```python
from build123d import *

# Parameters (mm, degrees)
SKETCH1_R             = 4
BOSS_EXTRUDE1_DEPTH   = 78.5
SKETCH2_R             = 2.5
BOSS_EXTRUDE2_DEPTH   = 8
CHAMFER1_SIZE         = 0.3
M4_TAPPED_HOLE1_D     = 3.3
M4_TAPPED_HOLE1_DEPTH = 10.1
M4_TAPPED_HOLE1_TIP   = 0.991420021
SKETCH6_R             = 1.75
CUT_EXTRUDE1_DEPTH    = 5
SKETCH7_W             = 0.3
SKETCH7_H             = 0.5


with BuildPart() as part:
    # Sketch1 → Boss-Extrude1 (new body)
    with BuildSketch(Plane(origin=(0, 0, 0), x_dir=(1, 0, 0), z_dir=(0, 1, 0))):
        with Locations(Location((0, 0, 0), (0, 0, 270))):
            Circle(SKETCH1_R)
    extrude(amount=BOSS_EXTRUDE1_DEPTH)

    # Sketch2 → Boss-Extrude2 (add)
    with BuildSketch(Plane(origin=(0, 78.5, 0), x_dir=(1, 0, 0), z_dir=(0, 1, 0))):
        with Locations(Location((0, 0, 0), (0, 0, 270))):
            Circle(SKETCH2_R)
    extrude(amount=BOSS_EXTRUDE2_DEPTH)

    # Chamfer1
    chamfer1_edges = [part.edges().sort_by_distance(p)[0] for p in [
        (0, 0, -4),
        (0, 78.5, -4),
        (0, 86.5, -2.5),
    ]]
    chamfer(chamfer1_edges, length=CHAMFER1_SIZE)

    # M4 Tapped Hole1
    with Locations(Plane(origin=(0, 0, 0), x_dir=(-1, 0, 0), z_dir=(0, -1, 0))):
        with Locations((0, 0)):
            Hole(M4_TAPPED_HOLE1_D / 2, depth=M4_TAPPED_HOLE1_DEPTH)
            with Locations((0, 0, -(M4_TAPPED_HOLE1_DEPTH + M4_TAPPED_HOLE1_TIP / 2))):  # 118° drill point
                Cone(0, M4_TAPPED_HOLE1_D / 2, M4_TAPPED_HOLE1_TIP, mode=Mode.SUBTRACT)

    # Sketch6 → Cut-Extrude1 (cut, symmetric)
    with BuildSketch(Plane.XY):
        with Locations(Location((0, 57, 0), (0, 0, 90))):
            Circle(SKETCH6_R)
    extrude(amount=CUT_EXTRUDE1_DEPTH, both=True, mode=Mode.SUBTRACT)

    # Sketch7 → Cut-Revolve1 (revolve, cut)
    with BuildSketch(Plane.XY, mode=Mode.PRIVATE) as cut_revolve1_sk:
        with Locations((2.35, 78.75)):
            Rectangle(SKETCH7_W, SKETCH7_H)
    revolve(cut_revolve1_sk.sketch.rotate(Axis((0, 0, 0), (0, 1, 0)), 90), axis=Axis((0, 0, 0), (0, 1, 0)), mode=Mode.SUBTRACT)


solid = part.part
```
Work out the finished part from the listing and answer in its coordinate system (mm). A direction names the side the tool comes from. Coordinates: 2 decimals unless noted, no trailing zeros. Loops run counter-clockwise (first coordinate to the right, second up) from the corner with the lowest first, then second, coordinate; pieces in that order, holes last. Notation, with made-up numbers: (87.25, 48.25) - (114.25, 48.25) arc R15 ccw to (114.25, 65.25) - close; hole circle Ø4 at (10.25, 28.5). An arc over 180 degrees is marked (long way). Use a Markdown table: item, result.
Item 1: The mould has two halves that part along Z. Classify faces 1 (the cylindrical face through (-2.44, 82.55, -0.54)), 2 (the flat face through (0, 86.5, 0)), 3 (the cylindrical face through (-1.216, 5.121, -1.115)): +Z half, -Z half, draft (parallel to the pull), parting line (faces both ways), or undercut.
Evaluation:
| item | result |
|---|---|
| face 1 | parting line |
| face 2 | draft |
| face 3 | undercut |
Item 2: Find section C-C, the plane y = 8. Determine the outline of the cut face in (x, z).
Evaluation:
| item | result |
|---|---|
| outline | circle Ø8 at (0, 0); hole circle Ø3.3 at (0, 0) |
Item 3: Find section B-B, the plane y = 57. Determine the outline of the cut face in (x, z).
Evaluation:
| item | result |
|---|---|
| outline | (-1.75, -3.6) - (-1.75, 3.6) arc R4 ccw to start; (1.75, -3.6) arc R4 ccw to (1.75, 3.6) - close |
Item 4: Given pin 1 Ø3 at (x, z) = (1.5, -2) entering from -Y; pin 2 Ø1.5 at (y, z) = (27.5, 3) entering from -X; pin 3 Ø1.5 at (x, y) = (-2.5, 47) entering from -Z, each flat-ended and moving along its own axis, determine where each tip first touches the part or whether it passes through.
Evaluation:
| item | result |
|---|---|
| pin 1 | stops at y = 0 |
| pin 2 | stops at x = -3.31 |
| pin 3 | stops at z = -3.6 |
Item 5: Consider probe 1 along Y at (x, z) = (0, 2.75); probe 2 along X at (y, z) = (57, 1.5); probe 3 along Z at (x, y) = (0, 7.25). Determine where each line is inside the solid, lowest interval first. Write a range as from..to.
Evaluation:
| item | result |
|---|---|
| probe 1 | y = 0..55.25, 58.75..78.5 |
| probe 2 | x = -3.71..-1.75, 1.75..3.71 |
| probe 3 | z = -4..-1.65, 1.65..4 |
Item 6: Find section A-A, the plane y = 72. Determine the outline of the cut face in (x, z), and give its area (3 significant figures).
Evaluation:
| item | result |
|---|---|
| outline | circle Ø8 at (0, 0) |
| area | 50.3 mm2 |
Item 7: For faces 4 (the cylindrical face through (-3.905, 38.705, -0.867)), 5 (the cylindrical face through (-2.18, 78.75, 0.29)), determine the directions among +Z, -Z, +X, -X, +Y, -Y from which every point of the face is accessible in a straight line to the end or side of a thin tool.
Evaluation:
| item | result |
|---|---|
| face 4 | +Y, -Y |
| face 5 | none |
